Job drawing, mm, ordinate dimensions from the low corner. One solid piece. A direction names the side the tool comes from. Coordinates: 2 decimals unless noted, no trailing zeros. Loops run counter-clockwise (first coordinate to the right, second up) from the corner with the lowest first, then second, coordinate; pieces in that order, holes last. Notation, with made-up numbers: M 66,-40 L 80,-40 A19 ccw 80,-6 Z; hole C 7,50.5 d4. An arc over 180 degrees is marked long. Write each question's results on one line, items separated by ' | '. Start each with the question number.
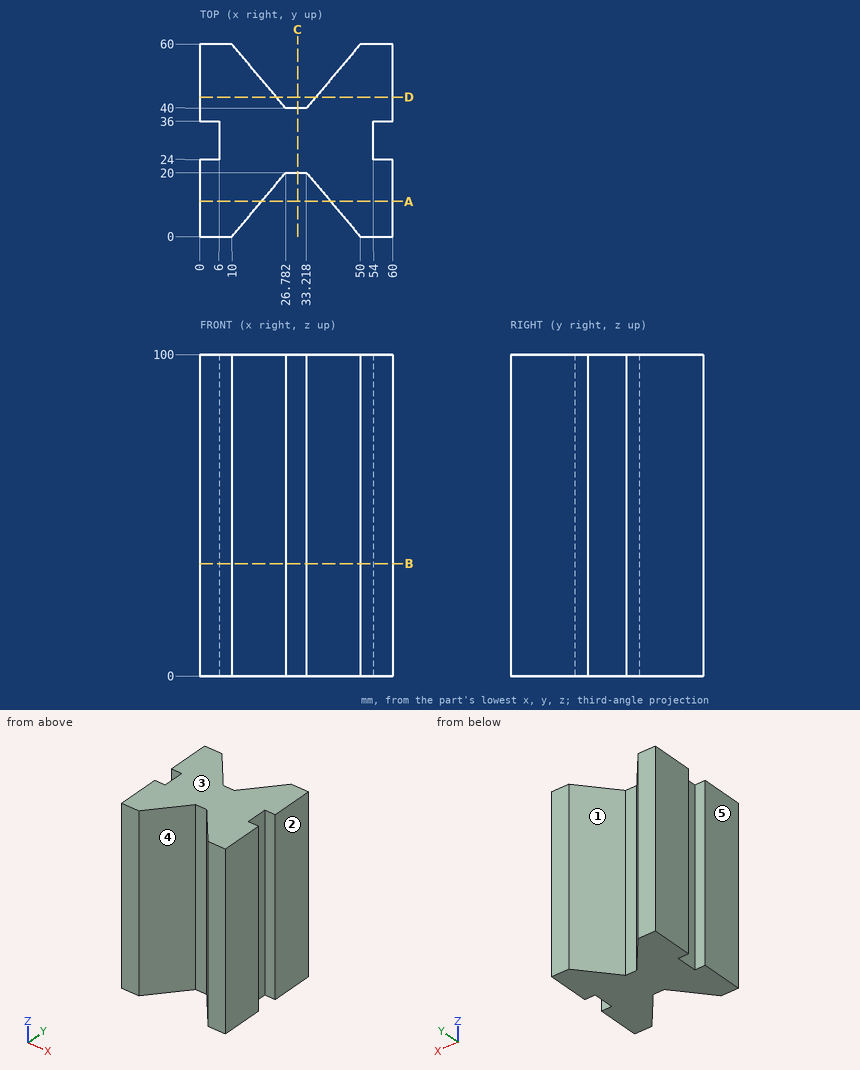
1. Band-saw the part on D-D, the plane y = 43.5. List the corners of the cut face in (x, z), plus the area to 3 significant figures.
2. Which spindle directions (+Z, -Z, +X, -X, +Y, -Y) get a long thin tool onto all of the face, cutting with end or side? Do the marked faces 4 and 5. Say none if no direction does.
3. Mould opens along X. For the marked faces 1, 2 and 3 say: +X half, -X half, draft (parallel to the pull), parting line (faces both ways), or undercut.
4. Band-saw the part on B-B, the plane z = 35. List the corners of the cut face in (x, y).
5. Wall check: line 1 along Y through (x, z) = (5, 35.5); line 2 along X through (y, z) = (47, 83); line 3 along X through (y, z) = (53.5, 77.5). Give the ranges that are in metal, low to high.
6. Band-saw the part on C-C, the plane x = 30.5. List the corners of the cut face in (y, z).
7. Pin check, flat tips, straight feed: pin 1 (7 mm diameter, centred on x = 30, z = 39, fed in from +Y); pin 2 (10 mm diameter, centred on x = 9, y = 16, fed in from -Z); pin 3 (8 mm diameter, centred on y = 31.5, z = 52, fed in from +X); pin 4 (3 mm diameter, centred on x = 23, z = 24, fed in from +Y). Stop position of each tip, or through.
8. Band-saw the part on A-A, the plane y = 11. List the corners of the cut face in (x, z), plus the area to 3 significant figures.
Checked values:
1) outline: M 0,0 L 23.85,0 L 23.85,100 L 0,100 Z; M 36.15,0 L 60,0 L 60,100 L 36.15,100 Z | area: 4,770 mm²
2) face 4: +Z, -Z, -Y | face 5: +Z, -Z, -X, +Y, -Y
3) face 1: undercut | face 2: +X half | face 3: draft
4) outline: M 0,0 L 10,0 L 26.78,20 L 33.22,20 L 50,0 L 60,0 L 60,24 L 54,24 L 54,36 L 60,36 L 60,60 L 50,60 L 33.22,40 L 26.78,40 L 10,60 L 0,60 L 0,36 L 6,36 L 6,24 L 0,24 Z
5) line 1: 0 to 24, 36 to 60 | line 2: 0 to 20.91, 39.09 to 60 | line 3: 0 to 15.45, 44.55 to 60
6) outline: M 20,0 L 40,0 L 40,100 L 20,100 Z
7) pin 1: y = 40.34 | pin 2: z = 0 | pin 3: x = 54 | pin 4: y = 46.29
8) outline: M 0,0 L 19.23,0 L 19.23,100 L 0,100 Z; M 40.77,0 L 60,0 L 60,100 L 40.77,100 Z | area: 3,850 mm²
